Answer from the drawing. Dimensions are ordinates in mm from the lowest x, y and z of the part. A direction names the side the tool comes from. Give positions to 0.01 mm unless a question says otherwise; leave off trailing zeros. Order: outer loops, then holes, each group sorted by start corner. A loop starts at its lowest first (then second) coordinate and runs counter-clockwise, first axis right, second up. Notation, with made-up numbers: (31.5, -27.5) - (45.5, -27.5) arc R16 ccw to (45.5, 2.5) - close; hole circle Ø8 at (31.25, 18.5). An arc over 180 degrees is marked (long way). Use a Markdown table: item, result. Add a question column.
1) Find section A-A, the plane y = 64. Determine the outline of the cut face in (x, z), plus the area to 3 significant figures.
2) Flat-ended cylindrical pins translate along their axes: pin 1 (3 mm diameter, centred on x = 9, z = 6, fed in from -Y); pin 2 (2 mm diameter, centred on x = 12, y = 49.5, fed in from -Z); pin 3 (6 mm diameter, centred on x = 29, y = 64, fed in from -Z). Find the tip coordinate at first contact, or state that the pin passes through.
3) For the marked faces 1 and 2, determine the directions among +Z, -Z, +X, -X, +Y, -Y from which every point of the face is accessible in a straight line to the end or side of a thin tool.
4) Find section C-C, the plane z = 9.5. Determine the outline of the cut face in (x, y), plus the area to 3 significant figures.
5) The mould has two halves that part along Y. Classify the marked faces 3, 4, 5 and 6: released by +Y, released by -Y, zero draft, split by the parting line, or undercut.
6) Find section B-B, the plane x = 9. Determine the outline of the cut face in (y, z), plus the area to 3 significant figures.
7) Straight lines are drawn through the part: line 1 (Z direction, x = 9, y = 7.75); line 2 (Y direction, x = 9, z = 5); line 3 (Y direction, x = 29, z = 2.5). For each, find the intervals that lie inside material, in ascending order.
8) Find section D-D, the plane y = 9.5. Determine the outline of the cut face in (x, z).
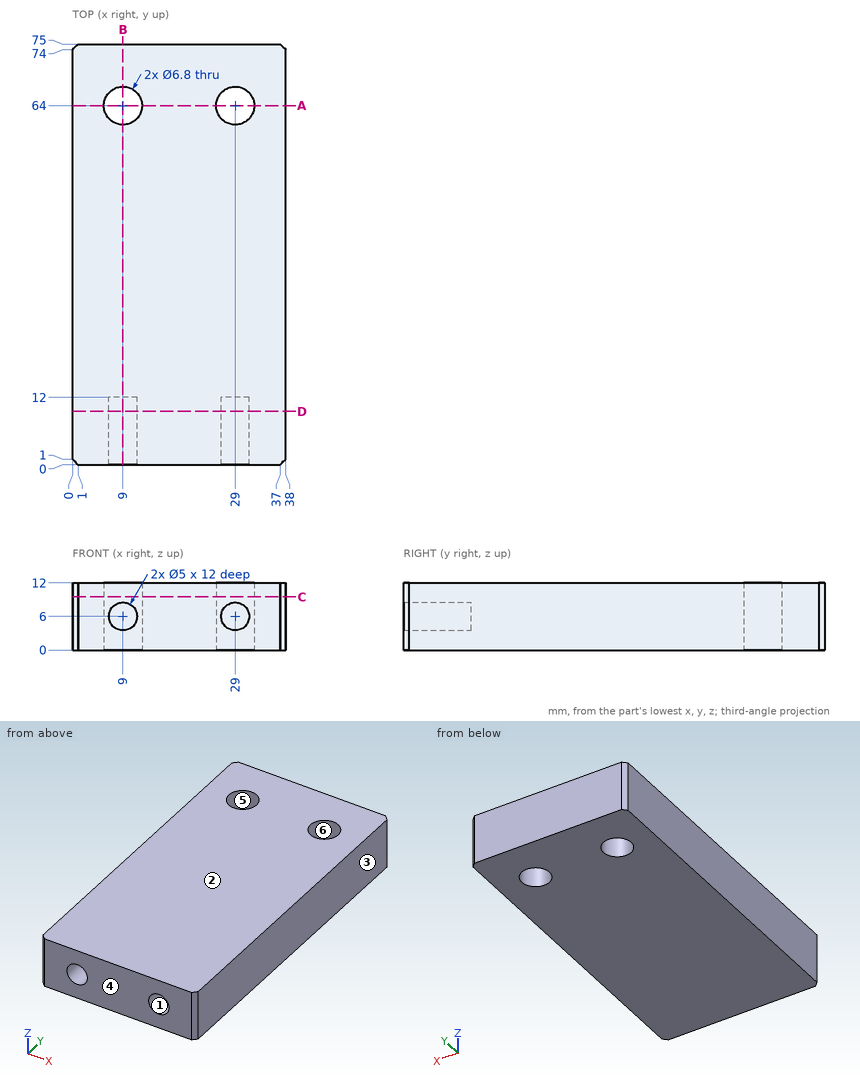
The answers:
| question | item | result |
|---|---|---|
| 1 | outline | (0, 0) - (5.6, 0) - (5.6, 12) - (0, 12) - close; (12.4, 0) - (25.6, 0) - (25.6, 12) - (12.4, 12) - close; (32.4, 0) - (38, 0) - (38, 12) - (32.4, 12) - close |
| 1 | area | 293 mm2 |
| 2 | pin 1 | y = 12 |
| 2 | pin 2 | z = 0 |
| 2 | pin 3 | through |
| 3 | face 1 | -Y |
| 3 | face 2 | +Z, +X, -X, +Y, -Y |
| 4 | outline | (0, 1) - (1, 0) - (37, 0) - (38, 1) - (38, 74) - (37, 75) - (1, 75) - (0, 74) - close; hole circle Ø6.8 at (9, 64); hole circle Ø6.8 at (29, 64) |
| 4 | area | 2,780 mm2 |
| 5 | face 3 | zero draft |
| 5 | face 4 | released by -Y |
| 5 | face 5 | undercut |
| 5 | face 6 | undercut |
| 6 | outline | (0, 0) - (60.6, 0) - (60.6, 12) - (0, 12) - (0, 8.5) - (12, 8.5) - (12, 3.5) - (0, 3.5) - close; (67.4, 0) - (75, 0) - (75, 12) - (67.4, 12) - close |
| 6 | area | 758 mm2 |
| 7 | line 1 | 0 to 3.5, 8.5 to 12 |
| 7 | line 2 | 12 to 60.6, 67.4 to 75 |
| 7 | line 3 | 0 to 60.6, 67.4 to 75 |
| 8 | outline | (0, 0) - (38, 0) - (38, 12) - (0, 12) - close; hole circle Ø5 at (9, 6); hole circle Ø5 at (29, 6) |
